The listing builds one solid part. Answer for the finished solid, in the listing's coordinates (mm). A direction names the side the tool comes from. Coordinates: 2 decimals unless noted, no trailing zeros. Loops run counter-clockwise (first coordinate to the right, second up) from the corner with the lowest first, then second, coordinate; pieces in that order, holes last. Notation, with made-up numbers: (79.25, 17.5) - (112.25, 17.5) arc R28 ccw to (112.25, 37.5) - close; hole circle Ø11 at (67, 83). An arc over 180 degrees is marked (long way). Return JSON: item names as keys, results as strings. Group by question number.
1. Which of the six approach directions +Z, -Z, +X, -X, +Y, -Y give full straight-line access (tool end or side, diameter ignored) to faces 4 (the face through (123, 17.5, 10)), 5 (the face through (43, 0, 0)), 6 (the face through (43, 0, -8)), 7 (the face through (129, -5, 5))?
2. Section A-A (x = 43) is taken. Write down the section's boundary in (y, z).
3. Find the intervals of material crossed by line 1 along Y through (x, z) = (11, -5); line 2 along X through (y, z) = (14, -7) (3 decimals); line 3 along Y through (x, z) = (124, 8), in increasing order.
4. Section C-C (y = -8) is taken. Write down the section's boundary in (x, z), and give its area (3 significant figures).
5. Each of these flat-tipped pins is pushed along its axis until it touches: P1, Ø12, axis at y = -6.5, z = 17, coming from the -X side; P2, Ø2, axis at x = 36.5, y = 20, coming from the -Z side; P3, Ø4, axis at x = 91, y = 2.5, coming from the +Z side. Where does it stop, or does it pass through?
6. Section D-D (z = 7.5) is taken. Write down the section's boundary in (x, y), and give its area (3 significant figures).
7. Section B-B (y = 16) is taken. Write down the section's boundary in (x, z), and give its area (3 significant figures).
8. The mould has two halves that part along Y. Classify faces 1 (the face through (123, -17.5, 10)), 2 (the face through (90, -27, 3)), 3 (the face through (92.79, 0.38, -3.61)): pulls with the +Y half, pulls with the -Y half, needs draft (parallel to the pull), parting line crosses it, or undercut.
```python
from build123d import *

# Parameters (mm, degrees)
BRACKET_BODY_DEPTH        = 27
PROFILE_TRIM_CUT_DEPTH    = 54
END_SLOT_CUT_DEPTH        = 60
MOUNTING_HOLES_SKETCH_R   = 3.5
MOUNTING_HOLES_6X_7_DEPTH = 8


with BuildPart() as part:
    # Bracket Profile Sketch → Bracket Body (new, symmetric)
    with BuildSketch(Plane(origin=(0, 0, 0), x_dir=(1, 0, 0), z_dir=(0, 1, 0))):
        Polygon((0, 0), (0, 8), (86.522390311, 8), (99.237588067, -0.903277318), (109.561963921, 13.841459479), (152.157870224, -15.984515211), (137.244882879, -37.282468363), (84, 0), align=None)
    extrude(amount=BRACKET_BODY_DEPTH, both=True)

    # Profile Trim Sketch → Profile Trim Cut (cut)
    with BuildSketch(Plane(origin=(42.548141325, 0, -60.765043225), x_dir=(-0.819152044288991, 0, -0.5735764363510474), z_dir=(0.5735764363510474, 0, -0.819152044288991))):
        with BuildLine():
            ThreePointArc((-133.80877172, 1.36e-07), (-131.883368797, 14.019084406), (-126.249743807, 27))
            Line((-126.249743807, 27), (-133.80877172, 27))
            Line((-133.80877172, 27), (-133.80877172, 1.36e-07))
        make_face()
        with BuildLine():
            ThreePointArc((-126.249743807, -27), (-131.883368834, -14.019084275), (-133.80877172, 1.36e-07))
            Line((-133.80877172, 1.36e-07), (-133.80877172, -27))
            Line((-133.80877172, -27), (-126.249743807, -27))
        make_face()
    extrude(amount=-PROFILE_TRIM_CUT_DEPTH, mode=Mode.SUBTRACT)

    # End Slot Sketch → End Slot Cut (cut)
    with BuildSketch(Plane(origin=(116.162945253, 0, 81.338169927), x_dir=(-0.5735764363510482, 0, 0.8191520442889904), z_dir=(-0.8191520442889904, 0, -0.5735764363510482))):
        Polygon((-74.180420653, 5), (-66.180420653, 5), (-66.180420653, 17.5), (-58.180420653, 17.5), (-58.180420653, -17.5), (-66.180420653, -17.5), (-66.180420653, -5), (-74.180420653, -5), align=None)
    extrude(amount=END_SLOT_CUT_DEPTH, mode=Mode.SUBTRACT)

    # Mounting Holes Sketch → Mounting Holes 6xØ7 (cut)
    with BuildSketch(Plane(origin=(0, 0, -8), x_dir=(-1, 0, 0), z_dir=(0, 0, -1))):
        with Locations((-11, 16)):
            Circle(MOUNTING_HOLES_SKETCH_R)
        with Locations((-11, -16)):
            Circle(MOUNTING_HOLES_SKETCH_R)
        with Locations((-43, 16)):
            Circle(MOUNTING_HOLES_SKETCH_R)
        with Locations((-43, -16)):
            Circle(MOUNTING_HOLES_SKETCH_R)
        with Locations((-75, 16)):
            Circle(MOUNTING_HOLES_SKETCH_R)
        with Locations((-75, -16)):
            Circle(MOUNTING_HOLES_SKETCH_R)
    extrude(amount=-MOUNTING_HOLES_6X_7_DEPTH, mode=Mode.SUBTRACT)


solid = part.part
```
The answers:
{
 "1": {"face 4": "none", "face 5": "+Z, -X, +Y, -Y", "face 6": "-Z, -X, +Y, -Y", "face 7": "-Z, +X"},
 "2": {"outline": "(-27, -8) - (-19.5, -8) - (-19.5, 0) - (-27, 0) - close; (-12.5, -8) - (12.5, -8) - (12.5, 0) - (-12.5, 0) - close; (19.5, -8) - (27, -8) - (27, 0) - (19.5, 0) - close"},
 "3": {"line 1": "y = -27 to -19.5, -12.5 to 12.5, 19.5 to 27", "line 2": "x = 0 to 8.128, 13.872 to 40.128, 45.872 to 72.128, 77.872 to 87.951, 105.385 to 119.333", "line 3": "y = -27 to -17.5, 17.5 to 27"},
 "4": {"outline": "(0, -8) - (86.52, -8) - (99.24, 0.9) - (100.38, -0.74) - (142.47, 28.74) - (136.74, 36.93) - (84, 0) - (0, 0) - close; (104.97, -7.29) - (109.56, -13.84) - (151.65, 15.63) - (147.06, 22.18) - close", "area": "1,720 mm2"},
 "5": {"P1": "stops at x = 99.71", "P2": "stops at z = -8", "P3": "stops at z = 6.3"},
 "6": {"outline": "(94.71, -27) - (140.04, -27) - (140.04, -5) - (126.09, -5) - (126.09, -17.5) - (112.15, -17.5) - (112.15, 17.5) - (126.09, 17.5) - (126.09, 5) - (140.04, 5) - (140.04, 27) - (94.71, 27) - close", "area": "1,820 mm2"},
 "7": {"outline": "(0, -8) - (7.5, -8) - (7.5, 0) - (0, 0) - close; (14.5, -8) - (39.5, -8) - (39.5, 0) - (14.5, 0) - close; (46.5, -8) - (71.5, -8) - (71.5, 0) - (46.5, 0) - close; (78.5, -8) - (86.52, -8) - (99.24, 0.9) - (100.38, -0.74) - (140.91, 27.64) - (135.18, 35.84) - (84, 0) - (78.5, 0) - close; (104.97, -7.29) - (109.56, -13.84) - (150.09, 14.54) - (145.5, 21.09) - close", "area": "1,520 mm2"},
 "8": {"face 1": "undercut", "face 2": "pulls with the -Y half", "face 3": "needs draft"}
}
